from build123d import *

# Parameters (mm, degrees)
SKETCH_2_W     = 2
SKETCH_2_H     = 4.343145751
CHAMFER_1_SIZE = 1.25


with BuildPart() as part:
    # 草图1 → 旋转1 (revolve)
    with BuildSketch(Plane(origin=(0, 0, 0), x_dir=(-1, 0, 0), z_dir=(0, 0, -1)), mode=Mode.PRIVATE) as revolve_1_sk:
        Polygon((-19.5, 6), (-19.5, 0), (19.5, 0), (19.5, 6), (-14.5, 6), (-14.5, 4.5), (-15.65, 4.5), (-15.65, 6), align=None)
    revolve(revolve_1_sk.sketch.rotate(Axis((19.5, 0, 0), (-1, 0, 0)), 270), axis=Axis((19.5, 0, 0), (-1, 0, 0)))

    # 草图2 → 旋转2 (revolve)
    with BuildSketch(Plane(origin=(-14.5, 0, 0), x_dir=(0, 0, -1), z_dir=(1, 0, 0))):
        with Locations((1, -7.828427125)):
            Rectangle(SKETCH_2_W, SKETCH_2_H)
    revolve(axis=Axis((-14.5, -5.656854249, 0), (0, -1, 0)))

    # 倒角1
    chamfer_1_edges = [part.edges().sort_by_distance(p)[0] for p in [
        (19.5, 0, -6),
        (-19.5, 0, -6),
    ]]
    chamfer(chamfer_1_edges, length=CHAMFER_1_SIZE)


solid = part.part
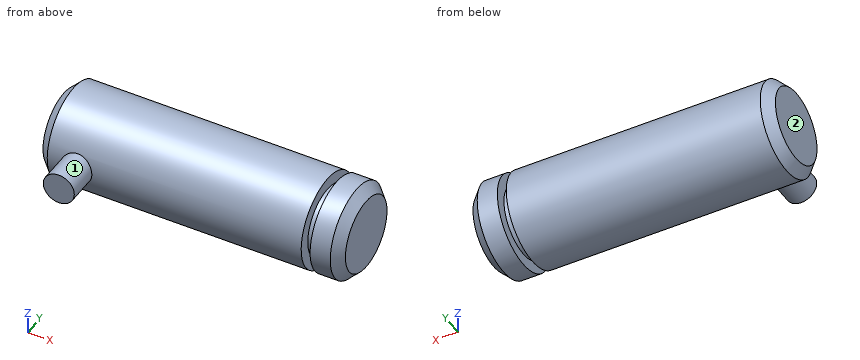
Model file for the job. Use its own axes, mm. Face numbers are marked on the shaded views. A direction names the side the tool comes from. Round coordinates to 2 decimals unless told otherwise and drop trailing zeros. Loops run counter-clockwise (first coordinate to the right, second up) from the corner with the lowest first, then second, coordinate; pieces in that order, holes last.
1. Tool access for the marked faces 1 and 2: list every direction of +Z, -Z, +X, -X, +Y, -Y with a clear straight run to the whole face (end or side of a thin tool).
Check values:
face 1: -Y
face 2: +Z, -Z, -X, +Y, -Y
2. Band-saw the part on A-A, the plane z = 0. List the corners of the cut face in (x, y), and give its area (3 significant figures).
Check values:
outline: (-19.5, -4.75) - (-18.25, -6) - (-16.5, -6) - (-16.5, -10) - (-12.5, -10) - (-12.5, -6) - (14.5, -6) - (14.5, -4.5) - (15.65, -4.5) - (15.65, -6) - (18.25, -6) - (19.5, -4.75) - (19.5, 4.75) - (18.25, 6) - (15.65, 6) - (15.65, 4.5) - (14.5, 4.5) - (14.5, 6) - (-18.25, 6) - (-19.5, 4.75) - close
area: 477 mm2
3. Band-saw the part on B-B, the plane x = -14.5. List the corners of the cut face in (y, z), and give its area (3 significant figures).
Check values:
outline: (-10, -2) - (-5.66, -2) arc R6 ccw (long way) to (-5.66, 2) - (-10, 2) - close
area: 130 mm2
4. Wall check: probe 1 along X at (y, z) = (1.75, 4.25); probe 2 along Y at (x, z) = (-13, -0.25); probe 3 along X at (y, z) = (-3.5, -4.25). Give the ranges that are in metal, low to high.
Check values:
probe 1: x = -19.5 to 14.5, 15.65 to 19.5
probe 2: y = -10 to 5.99
probe 3: x = -18.74 to 14.5, 15.65 to 18.74
5. Drop flat-ended pins along their axis: P1, Ø1, axis at x = -12.5, z = 3, coming from the -Y side; P2, Ø5, axis at y = -8.5, z = -3, coming from the +X side; P3, Ø6, axis at x = -8, z = -4.5, coming from the +Y side; P4, Ø5, axis at x = 12.5, z = -1.5, coming from the +Y side. Give the stop position or say it passes through.
Check values:
P1: stops at y = -5.45
P2: stops at x = -12.56
P3: stops at y = 5.81
P4: stops at y = 6
